Geometry check sheet. Reference: the model listing, model coordinates, mm. Face numbers are marked on the shaded views. A direction names the side the tool comes from. Give positions to 0.01 mm unless a question says otherwise; leave off trailing zeros. Order: outer loops, then holes, each group sorted by start corner. A loop starts at its lowest first (then second) coordinate and runs counter-clockwise, first axis right, second up.
from build123d import *

# Parameters (mm, degrees)
BASE_PLATE_PROFILE_SKETCH_R = 10
BASE_PLATE_30MM_DEPTH       = 30
POCKET_25MM_DEEP_DEPTH      = 25


with BuildPart() as part:
    # Base Plate Profile Sketch → Base Plate 30mm (new body)
    with BuildSketch(Plane(origin=(0, 0, 0), x_dir=(1, 0, 0), z_dir=(0, 1, 0))):
        with BuildLine():
            Line((-74.980820796, 1.369858652), (-4.980820796, 19.369858652))
            ThreePointArc((-4.980820796, 19.369858652), (0, 20), (4.980820796, 19.369858652))
            Line((4.980820796, 19.369858652), (74.980820796, 1.369858652))
            ThreePointArc((74.980820796, 1.369858652), (85.80532214, -5.74472391), (90, -18))
            Line((90, -18), (90, -88))
            ThreePointArc((90, -88), (80.846522891, -104.803361008), (61.764705882, -106.225803982))
            ThreePointArc((61.764705882, -106.225803982), (0, -92.919333848), (-61.764705882, -106.225803982))
            ThreePointArc((-61.764705882, -106.225803982), (-80.846522891, -104.803361008), (-90, -88))
            Line((-90, -88), (-90, -18))
            ThreePointArc((-90, -18), (-85.80532214, -5.74472391), (-74.980820796, 1.369858652))
        make_face()
        with Locations(Location((0, 0, 0), (0, 0, 270))):
            Circle(BASE_PLATE_PROFILE_SKETCH_R, mode=Mode.SUBTRACT)
        with Locations(Location((-70, -88, 0), (0, 0, 270))):
            Circle(BASE_PLATE_PROFILE_SKETCH_R, mode=Mode.SUBTRACT)
        with Locations(Location((70, -88, 0), (0, 0, 270))):
            Circle(BASE_PLATE_PROFILE_SKETCH_R, mode=Mode.SUBTRACT)
    extrude(amount=BASE_PLATE_30MM_DEPTH)

    # Pocket Profile Sketch → Pocket 25mm Deep (cut)
    with BuildSketch(Plane(origin=(0, 30, 0), x_dir=(1, 0, 0), z_dir=(0, 1, 0))):
        with BuildLine():
            Line((-85, -18), (-85, -70.679491924))
            ThreePointArc((-85, -70.679491924), (-82.5, -75.009618943), (-77.5, -75.009618943))
            ThreePointArc((-77.5, -75.009618943), (-61.541849411, -75.612115249), (-55.170564121, -90.255622199))
            ThreePointArc((-55.170564121, -90.255622199), (-53.453138568, -94.827801509), (-48.657811989, -95.75474119))
            ThreePointArc((-48.657811989, -95.75474119), (0, -87.919333848), (48.657811989, -95.75474119))
            ThreePointArc((48.657811989, -95.75474119), (53.453138568, -94.827801509), (55.170564121, -90.255622199))
            ThreePointArc((55.170564121, -90.255622199), (61.541849411, -75.612115249), (77.5, -75.009618943))
            ThreePointArc((77.5, -75.009618943), (82.5, -75.009618943), (85, -70.679491924))
            Line((85, -70.679491924), (85, -18))
            ThreePointArc((85, -18), (81.853991605, -8.808542933), (73.735615597, -3.472606011))
            Line((73.735615597, -3.472606011), (20.510405257, 10.213876648))
            ThreePointArc((20.510405257, 10.213876648), (15.694105243, 8.871023652), (14.448900044, 4.028558989))
            ThreePointArc((14.448900044, 4.028558989), (0, -15), (-14.448900044, 4.028558989))
            ThreePointArc((-14.448900044, 4.028558989), (-15.694105243, 8.871023652), (-20.510405257, 10.213876648))
            Line((-20.510405257, 10.213876648), (-73.735615597, -3.472606011))
            ThreePointArc((-73.735615597, -3.472606011), (-81.853991605, -8.808542933), (-85, -18))
        make_face()
    extrude(amount=-POCKET_25MM_DEEP_DEPTH, mode=Mode.SUBTRACT)


solid = part.part
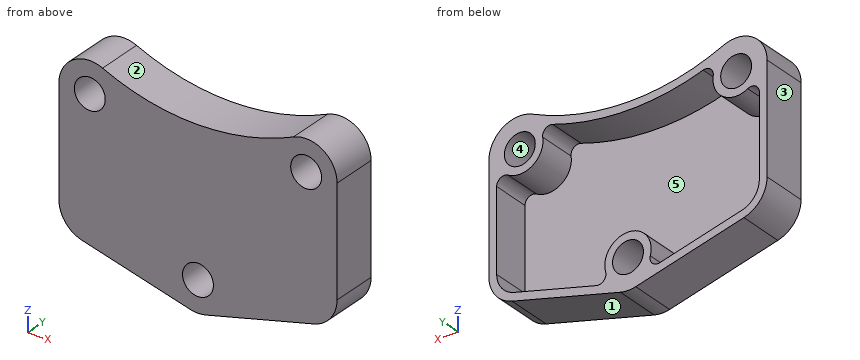
Item 1: Sectioned sample at B-B (x = 0). Enter the section's corners in (y, z), and give its area (3 significant figures).
Reported:
outline: (0, -20) - (30, -20) - (30, -10) - (0, -10) - close; (0, 10) - (30, 10) - (30, 15) - (5, 15) - (5, 87.92) - (30, 87.92) - (30, 92.92) - (0, 92.92) - close
area: 965 mm2
Item 2: Sectioned sample at D-D (x = 52.5). Enter the section's corners in (y, z), and give its area (3 significant figures).
Reported:
outline: (0, -7.15) - (30, -7.15) - (30, -1.99) - (5, -1.99) - (5, 95.46) - (30, 95.46) - (30, 102.41) - (0, 102.41) - close
area: 850 mm2
Item 3: Scan lines: L1, parallel to X at y = 14, z = 41.5; L2, parallel to Y at x = 68.5, z = 16; L3, parallel to Z at x = 72, y = 28.75. Record each from-to range of solid material in increasing order.
Reported:
L1: x = -90 to -85, 85 to 90
L2: y = 0 to 5
L3: z = -2.14 to 3.03, 73.13 to 78.2, 97.8 to 107.9
Item 4: Sectioned sample at C-C (z = 62). Enter the section's corners in (x, y).
Reported:
outline: (-90, 0) - (90, 0) - (90, 30) - (85, 30) - (85, 5) - (-85, 5) - (-85, 30) - (-90, 30) - close
Item 5: Gauge pin test, flat ends, axial feed: pin 1 (10 mm diameter, centred on x = -1, z = 39.5, fed in from -Y); pin 2 (3 mm diameter, centred on x = 5, z = 16.5, fed in from +Y); pin 3 (4 mm diameter, centred on x = 58, y = 6, fed in from -Z); pin 4 (4 mm diameter, centred on x = -21, y = 23, fed in from +Z). Record the tip position at first contact, or that the pin passes through.
Reported:
pin 1: stops at y = 0
pin 2: stops at y = 5
pin 3: stops at z = -6.25
pin 4: stops at z = 94.69
Item 6: Sectioned sample at A-A (y = 2.25). Enter the section's corners in (x, z).
Reported:
outline: (-90, 18) arc R20 ccw to (-74.98, -1.37) - (-4.98, -19.37) arc R20 ccw to (4.98, -19.37) - (74.98, -1.37) arc R20 ccw to (90, 18) - (90, 88) arc R20 ccw to (61.76, 106.23) arc R150 cw to (-61.76, 106.23) arc R20 ccw to (-90, 88) - close; hole circle Ø20 at (-70, 88); hole circle Ø20 at (0, 0); hole circle Ø20 at (70, 88)
Item 7: Set-up check for the marked faces 4 and 5: record each of +Z, -Z, +X, -X, +Y, -Y from which the full face is reachable in a straight line by a thin tool's end or side.
Reported:
face 4: +Y, -Y
face 5: +Y
Item 8: Draft check along X on the marked faces 1, 2 and 3. Enter one of: released by +X, released by -X, zero draft, split by the parting line, or undercut.
Reported:
face 1: released by +X
face 2: undercut
face 3: released by -X
